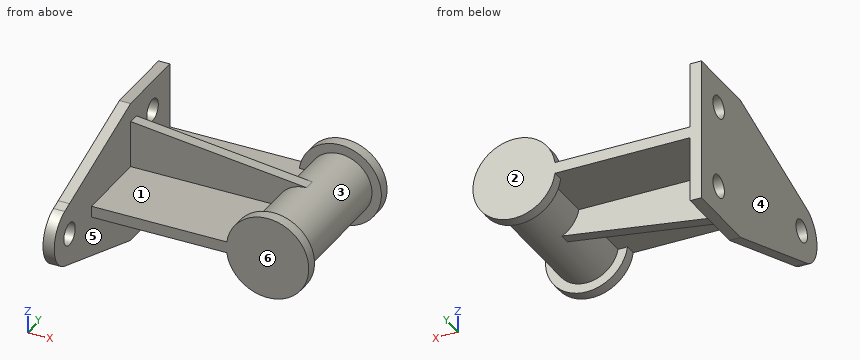
from build123d import *

# Parameters (mm, degrees)
POST_34_DEPTH              = 82
SKETCH1_4_R                = 22
SKETCH1_4_R_2              = 17
BASE_COLLAR_44_DEPTH       = 6
TOP_START                  = -6
TOP_CAP_SKETCH_R           = 22
TOP_CAP_SKETCH_R_2         = 17
TOP_CAP_DEPTH              = 6
SUPPORT_ARM_PROFILE_W      = 94
SUPPORT_ARM_PROFILE_H      = 3
SUPPORT_ARM_PROFILE_W_2    = 6
SUPPORT_ARM_PROFILE_H_2    = 35
SUPPORT_ARM_DEPTH          = 41
WALL_START                 = -6
WALL_PLATE_DEPTH           = 6
LOWER_PLATE_LOBE_SKETCH_R  = 6
LOWER_PLATE_LOBE_DEPTH     = 6
MOUNTING_HOLES_SKETCH_R    = 6
MOUNTING_HOLES_2X_12_DEPTH = 6
STIFFENER_RIB_SKETCH_W     = 94
STIFFENER_RIB_SKETCH_H     = 6
STIFFENER_RIB_DEPTH        = 41


with BuildPart() as part:
    # Post and Collar Profile → Post _34 (new body)
    with BuildSketch(Plane(origin=(0, 0, 0), x_dir=(1, 0, 0), z_dir=(0, 1, 0))):
        with BuildLine():
            ThreePointArc((17, 0), (0, 17), (-17, 0))
            Line((-17, 0), (17, 0))
        make_face()
        with BuildLine():
            Line((17, 0), (-17, 0))
            ThreePointArc((-17, 0), (0, -17), (17, 0))
        make_face()
        with BuildLine():
            ThreePointArc((17, 0), (0, 17), (-17, 0))
            Line((-17, 0), (17, 0))
        make_face()
        with BuildLine():
            Line((17, 0), (-17, 0))
            ThreePointArc((-17, 0), (0, -17), (17, 0))
        make_face()
    extrude(amount=POST_34_DEPTH)

    # Sketch1_4 → Base Collar _44 (add)
    with BuildSketch(Plane(origin=(0, 0, 0), x_dir=(1, 0, 0), z_dir=(0, 1, 0))):
        with Locations(Location((0, 0, 0), (0, 0, 270))):
            Circle(SKETCH1_4_R)
        with Locations(Location((0, 0, 0), (0, 0, 270))):
            Circle(SKETCH1_4_R_2, mode=Mode.SUBTRACT)
    extrude(amount=BASE_COLLAR_44_DEPTH)

    # Top Cap Sketch → Top Cap (add)
    with BuildSketch(Plane(origin=(0, 82, 0), x_dir=(1, 0, 0), z_dir=(0, 1, 0)).offset(TOP_START)):
        with Locations(Location((0, 0, 0), (0, 0, 270))):
            Circle(TOP_CAP_SKETCH_R)
        with Locations(Location((0, 0, 0), (0, 0, 270))):
            Circle(TOP_CAP_SKETCH_R_2, mode=Mode.SUBTRACT)
    extrude(amount=TOP_CAP_DEPTH)

    # Support Arm Profile → Support Arm (add)
    with BuildSketch(Plane(origin=(0, 82, 0), x_dir=(1, 0, 0), z_dir=(0, 1, 0))):
        with Locations((-47, -1.5)):
            Rectangle(SUPPORT_ARM_PROFILE_W, SUPPORT_ARM_PROFILE_H)
        with Locations((-47, 1.5)):
            Rectangle(SUPPORT_ARM_PROFILE_W, SUPPORT_ARM_PROFILE_H)
        with Locations((-97, -20.5)):
            Rectangle(SUPPORT_ARM_PROFILE_W_2, SUPPORT_ARM_PROFILE_H_2)
        with Locations((-97, -1.5)):
            Rectangle(SUPPORT_ARM_PROFILE_W_2, SUPPORT_ARM_PROFILE_H)
        with Locations((-97, 1.5)):
            Rectangle(SUPPORT_ARM_PROFILE_W_2, SUPPORT_ARM_PROFILE_H)
        with Locations((-97, 20.5)):
            Rectangle(SUPPORT_ARM_PROFILE_W_2, SUPPORT_ARM_PROFILE_H_2)
    extrude(amount=-SUPPORT_ARM_DEPTH)

    # Wall Plate Sketch → Wall Plate (add)
    with BuildSketch(Plane(origin=(0, 47, 0), x_dir=(1, 0, 0), z_dir=(0, 1, 0)).offset(WALL_START)):
        with BuildLine():
            Line((-16.733200531, -3), (-94, -3))
            Line((-94, -3), (-94, -28))
            Line((-94, -28), (0, -17))
            ThreePointArc((0, -17), (-10.908712115, -13.03840481), (-16.733200531, -3))
        make_face()
        with BuildLine():
            Line((-94, 3), (-16.733200531, 3))
            ThreePointArc((-16.733200531, 3), (-13.649862572, 10.133175798), (-7.714262086, 15.148932651))
            Line((-7.714262086, 15.148932651), (-94, 28))
            Line((-94, 28), (-94, 3))
        make_face()
    extrude(amount=WALL_PLATE_DEPTH)

    # Lower Plate Lobe Sketch → Lower Plate Lobe (add)
    with BuildSketch(Plane.ZY.offset(100)):
        with BuildLine():
            Line((38, 41), (-38, 41))
            Line((-38, 41), (-15.192006216, -28.020253691))
            ThreePointArc((-15.192006216, -28.020253691), (0, -39), (15.192006216, -28.020253691))
            Line((15.192006216, -28.020253691), (16.850967302, -23))
            Line((16.850967302, -23), (38, 41))
        make_face()
        with Locations((0, -23)):
            Circle(LOWER_PLATE_LOBE_SKETCH_R, mode=Mode.SUBTRACT)
    extrude(amount=-LOWER_PLATE_LOBE_DEPTH)

    # Mounting Holes Sketch → Mounting Holes 2x_12 (cut)
    with BuildSketch(Plane.ZY.offset(100)):
        with Locations((-22, 64)):
            Circle(MOUNTING_HOLES_SKETCH_R)
        with Locations((22, 64)):
            Circle(MOUNTING_HOLES_SKETCH_R)
    extrude(amount=-MOUNTING_HOLES_2X_12_DEPTH, mode=Mode.SUBTRACT)

    # Stiffener Rib Sketch → Stiffener Rib (add)
    with BuildSketch(Plane.XZ):
        with Locations((-47, 0)):
            Rectangle(STIFFENER_RIB_SKETCH_W, STIFFENER_RIB_SKETCH_H)
    extrude(amount=-STIFFENER_RIB_DEPTH)


solid = part.part
Read the model definition and answer for the solid it produces. Units are mm, in the model's axes. Face numbers are marked on the shaded views. A direction names the side the tool comes from. Coordinates: 2 decimals unless noted, no trailing zeros. Loops run counter-clockwise (first coordinate to the right, second up) from the corner with the lowest first, then second, coordinate; pieces in that order, holes last. Notation, with made-up numbers: (-25, 18.25) - (20, 18.25) arc R22 ccw to (20, 42.25) - close; hole circle Ø5 at (40.25, 89.5). An arc over 180 degrees is marked (long way). Answer in a Markdown table with one row per item.
Q1. For the marked faces 5 and 6, determine the directions among +Z, -Z, +X, -X, +Y, -Y from which every point of the face is accessible in a straight line to the end or side of a thin tool.
Here are the results:
| item | result |
|---|---|
| face 5 | none |
| face 6 | +Z, -Z, +X, -Y |
Q2. Given P1, Ø7, axis at y = -23, z = 0, coming from the -X side; P2, Ø8, axis at x = -86.5, y = 4.5, coming from the +Z side; P3, Ø13, axis at x = -38.5, z = -5.5, coming from the -Y side; P4, Ø12.5, axis at x = -55, z = 10, coming from the +Y side, each flat-ended and moving along its own axis, determine where each tip first touches the part or whether it passes through.
Here are the results:
| item | result |
|---|---|
| P1 | passes through |
| P2 | stops at z = 3 |
| P3 | stops at y = 0 |
| P4 | stops at y = 47 |
Q3. The mould has two halves that part along X. Classify the marked faces 1, 2, 3 and 4: pulls with the +X half, pulls with the -X half, needs draft (parallel to the pull), parting line crosses it, or undercut.
Here are the results:
| item | result |
|---|---|
| face 1 | undercut |
| face 2 | needs draft |
| face 3 | undercut |
| face 4 | pulls with the -X half |
Q4. Find section D-D on y = 27. Write down the section's boundary in (x, z), plus the area to 3 significant figures.
Here are the results:
| item | result |
|---|---|
| outline | (-100, -33.37) - (-94, -33.37) - (-94, -3) - (-16.73, -3) arc R17 ccw (long way) to (-16.73, 3) - (-94, 3) - (-94, 33.37) - (-100, 33.37) - close |
| area | 1,770 mm^2 |
Q5. Find section B-B on y = 64. Write down the section's boundary in (x, z), plus the area to 3 significant figures.
Here are the results:
| item | result |
|---|---|
| outline | (-100, -38) - (-94, -38) - (-94, -28) - (-100, -28) - close; (-100, -16) - (-94, -16) - (-94, -3) - (-16.73, -3) arc R17 ccw (long way) to (-16.73, 3) - (-94, 3) - (-94, 16) - (-100, 16) - close; (-100, 28) - (-94, 28) - (-94, 38) - (-100, 38) - close |
| area | 1,680 mm^2 |
Q6. Straight lines are drawn through the part: line 1 along Y through (x, z) = (-51.5, -16); line 2 along X through (y, z) = (58, 8); line 3 along X through (y, z) = (50.5, 24). For each, find the intervals that lie inside material, in ascending order. Write a range as [from, to].
Here are the results:
| item | result |
|---|---|
| line 1 | y = [41, 47] |
| line 2 | x = [-100, -94], [-15, 15] |
| line 3 | x = [-100, -94] |
Q7. Find section A-A on z = 0. Write down the section's boundary in (x, y), plus the area to 3 significant figures.
Here are the results:
| item | result |
|---|---|
| outline | (-100, -39) - (-94, -39) - (-94, -29) - (-100, -29) - close; (-100, -17) - (-94, -17) - (-94, 0) - (22, 0) - (22, 6) - (17, 6) - (17, 76) - (22, 76) - (22, 82) - (-100, 82) - close |
| area | 9,820 mm^2 |
Q8. Find section C-C on x = 12.5. Write down the section's boundary in (y, z), plus the area to 3 significant figures.
Here are the results:
| item | result |
|---|---|
| outline | (0, -18.1) - (6, -18.1) - (6, -11.52) - (76, -11.52) - (76, -18.1) - (82, -18.1) - (82, 18.1) - (76, 18.1) - (76, 11.52) - (6, 11.52) - (6, 18.1) - (0, 18.1) - close |
| area | 2,050 mm^2 |
